Verification items for this drawing (mm, ordinates from the low corner). A direction names the side the tool comes from. Round coordinates to 2 decimals unless told otherwise and drop trailing zeros. Order: outer loops, then holes, each group sorted by start corner. A loop starts at its lowest first (then second) coordinate and runs counter-clockwise, first axis right, second up. Notation, with made-up numbers: (47, 56.25) - (82, 56.25) arc R30 cw to (82, 83.25) - close; hole circle Ø6 at (-24, 5.5). An arc over 180 degrees is marked (long way). Return JSON: item names as keys, results as strings. Group by question number.
Q1. Tool access check on the marked faces 1, 2 and 3. Record the directions out of +Z, -Z, +X, -X, +Y, -Y that give a thin tool (end or side, any length) a straight path to the whole face; none if there is none.
Q2. Gauge pin test, flat end, axial feed: pin 1 Ø2 at (y, z) = (4.5, 9) entering from -X. Record the tip position at first contact, or that the pin passes through.
Q3. Sectioned sample at A-A, the plane z = 1.25. Record the cut outline in (x, y).
Q4. Sectioned sample at B-B, the plane z = 9.25. Record the cut outline in (x, y), then the cut area to 3 significant figures.
Q5. Material ranges on line 1 along Z through (x, y) = (1.3, 2.65); line 2 along Z through (x, y) = (0.3, 1.6); line 3 along Y through (x, z) = (2.55, 8.25), recorded low to high.
Q6. Sectioned sample at C-C, the plane z = 4.25. Record the cut outline in (x, y).
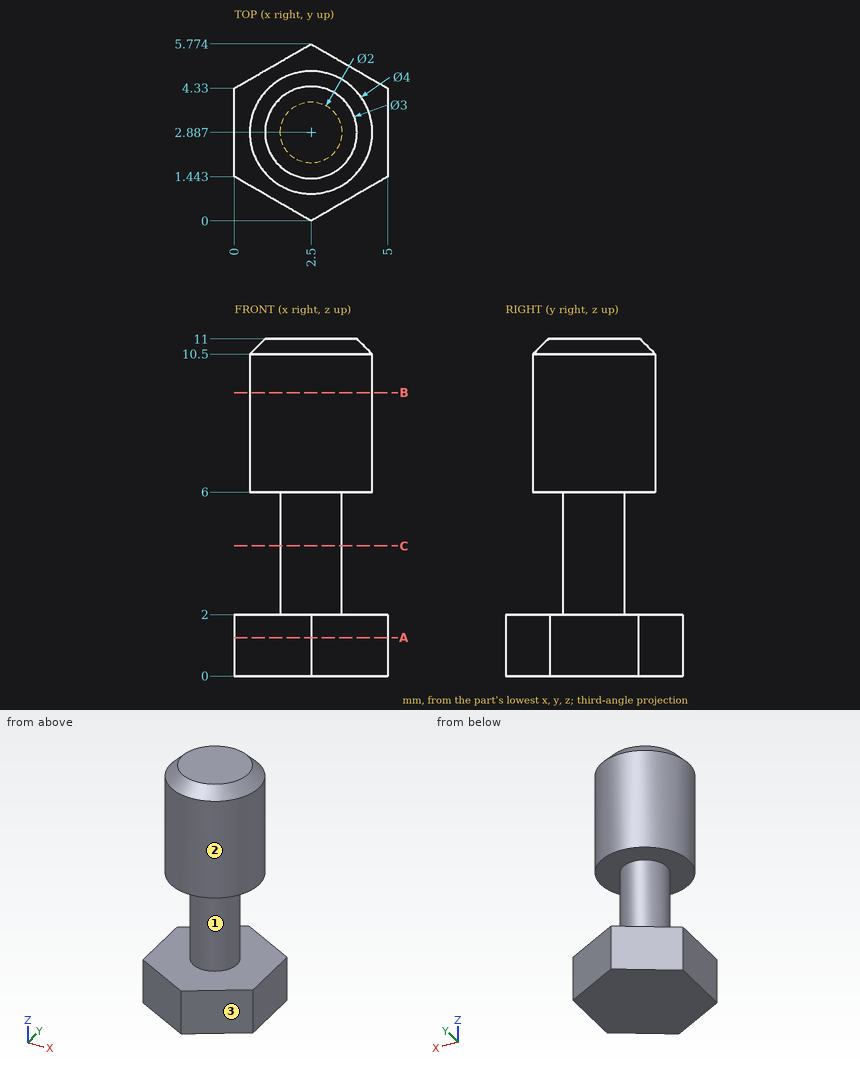
Reply:
{
 "1": {"face 1": "none", "face 2": "+Z", "face 3": "+Z, -Z, +X, -Y"},
 "2": {"pin 1": "x = 0.6"},
 "3": {"outline": "(0, 1.44) - (2.5, 0) - (5, 1.44) - (5, 4.33) - (2.5, 5.77) - (0, 4.33) - close"},
 "4": {"outline": "circle Ø4 at (2.5, 2.89)", "area": "12.6 mm^2"},
 "5": {"line 1": "0 to 2, 6 to 11", "line 2": "0 to 2", "line 3": "0.89 to 4.89"},
 "6": {"outline": "circle Ø2 at (2.5, 2.89)"}
}
